The listing builds one solid part. Answer for the finished solid, in the listing's coordinates (mm). A direction names the side the tool comes from. Give positions to 0.01 mm unless a question says otherwise; leave off trailing zeros. Write each loop counter-clockwise with the first axis right and the second up, starting at its lowest first coordinate (ties: lowest second). Pieces come first, ordered by that corner, then holes. Notation, with made-up numbers: M 8.5,40 L 65.5,40 A19 ccw 65.5,66 Z; hole C 46,41.5 d7. An arc over 180 degrees is marked long. Return JSON: item names as keys, results as strings.
from build123d import *

# Parameters (mm, degrees)
FLANGE_PROFILE_R       = 12.5
FLANGE_PROFILE_R_2     = 12.920835642
FLANGE_PLATE_DEPTH     = 5
HUB_PROFILE_R          = 25
HUB_PROFILE_R_2        = 15
HUB_50_BORE_30_DEPTH   = 60
CROSS_SLOT_PROFILE_W   = 10
CROSS_SLOT_PROFILE_H   = 10.92
CROSS_SLOT_PROFILE_W_2 = 10.92
CROSS_SLOT_PROFILE_H_2 = 10
CROSS_SLOTS_4X10_DEPTH = 5


with BuildPart() as part:
    # Flange Profile → Flange Plate (new, symmetric)
    with BuildSketch(Plane(origin=(0, 0, 0), x_dir=(1, 0, 0), z_dir=(0, 1, 0))):
        with BuildLine():
            Line((-62.717391304, 19.30748114), (-9.130434783, 33.788091995))
            ThreePointArc((-9.130434783, 33.788091995), (0.242124563, 34.9991625), (9.597031237, 33.658535195))
            Line((9.597031237, 33.658535195), (57.5, 20))
            ThreePointArc((57.5, 20), (77.5, 0), (57.5, -20))
            Line((57.5, -20), (9.597031237, -33.658535195))
            ThreePointArc((9.597031237, -33.658535195), (0.242124563, -34.9991625), (-9.130434783, -33.788091995))
            Line((-9.130434783, -33.788091995), (-62.717391304, -19.30748114))
            ThreePointArc((-62.717391304, -19.30748114), (-77.5, 0), (-62.717391304, 19.30748114))
        make_face()
        with Locations(Location((-57.5, 0, 0), (0, 0, 270))):
            Circle(FLANGE_PROFILE_R, mode=Mode.SUBTRACT)
        with Locations(Location((57.5, 0, 0), (0, 0, 270))):
            Circle(FLANGE_PROFILE_R_2, mode=Mode.SUBTRACT)
    extrude(amount=FLANGE_PLATE_DEPTH, both=True)

    # Hub Profile → Hub Ø50 Bore Ø30 (add)
    with BuildSketch(Plane(origin=(0, 5, 0), x_dir=(1, 0, 0), z_dir=(0, 1, 0))):
        with Locations(Location((0, 0, 0), (0, 0, 270))):
            Circle(HUB_PROFILE_R)
        with Locations(Location((0, 0, 0), (0, 0, 270))):
            Circle(HUB_PROFILE_R_2, mode=Mode.SUBTRACT)
    extrude(amount=HUB_50_BORE_30_DEPTH)

    # Cross Slot Profile → Cross Slots 4x10 (cut)
    with BuildSketch(Plane(origin=(0, 65, 0), x_dir=(1, 0, 0), z_dir=(0, 1, 0))):
        with Locations((0, 19.602135624)):
            Rectangle(CROSS_SLOT_PROFILE_W, CROSS_SLOT_PROFILE_H)
        with Locations((19.602135624, 0)):
            Rectangle(CROSS_SLOT_PROFILE_W_2, CROSS_SLOT_PROFILE_H_2)
        with Locations((0, -19.602135624)):
            Rectangle(CROSS_SLOT_PROFILE_W, CROSS_SLOT_PROFILE_H)
        with Locations((-19.602135624, 0)):
            Rectangle(CROSS_SLOT_PROFILE_W_2, CROSS_SLOT_PROFILE_H_2)
    extrude(amount=-CROSS_SLOTS_4X10_DEPTH, mode=Mode.SUBTRACT)


solid = part.part
Item 1: A cutting plane is placed at C-C, the plane x = -57.5. Write down the section's boundary in (y, z).
Geometry results:
{"outline": "M -5,-20.72 L 5,-20.72 L 5,-12.5 L -5,-12.5 Z; M -5,12.5 L 5,12.5 L 5,20.72 L -5,20.72 Z"}
Item 2: Find the intervals of material crossed by line 1 (X direction, y = -3, z = 0); line 2 (X direction, y = 34, z = 0); line 3 (X direction, y = -1.5, z = 7.5), in increasing order.
Geometry results:
{"line 1": "x = -77.5 to -70, -45 to 44.58, 70.42 to 77.5", "line 2": "x = -25 to -15, 15 to 25", "line 3": "x = -76.04 to -67.5, -47.5 to 46.98, 68.02 to 76.04"}
Item 3: Given pin 1 Ø5.5 at (x, y) = (-20, 63) entering from +Z; pin 2 Ø4 at (y, z) = (63.5, 21) entering from -X; pin 3 Ø4 at (y, z) = (63, 19.5) entering from +X; pin 4 Ø3 at (x, z) = (-9.5, 10) entering from +Y, each flat-ended and moving along its own axis, determine where each tip first touches the part or whether it passes through.
Geometry results:
{"pin 1": "stops at z = 18.1", "pin 2": "stops at x = -16.25", "pin 3": "stops at x = 17.85", "pin 4": "stops at y = 65"}
Item 4: A cutting plane is placed at D-D, the plane y = 35. Write down the section's boundary in (x, z), plus the area to 3 significant figures.
Geometry results:
{"outline": "C 0,0 d50; hole C 0,0 d30", "area": "1,260 mm2"}
Item 5: Which of the six approach directions +Z, -Z, +X, -X, +Y, -Y give full straight-line access (tool end or side, diameter ignored) to faces 4 (the cylindrical face through (-13.31, 34.58, 6.92)), 5 (the cylindrical face through (-45.106, -0.07, -1.627)), 6 (the flat face through (0, 60, -20))?
Geometry results:
{"face 4": "+Y", "face 5": "+Y, -Y", "face 6": "+Z, -Z, +Y"}
Item 6: A cutting plane is placed at A-A, the plane y = 1.5. Write down the section's boundary in (x, z).
Geometry results:
{"outline": "M -62.72,-19.31 L -9.13,-33.79 A35 ccw 9.6,-33.66 L 57.5,-20 A20 ccw 57.5,20 L 9.6,33.66 A35 ccw -9.13,33.79 L -62.72,19.31 A20 ccw Z; hole C -57.5,0 d25; hole C 57.5,0 d25.84"}
Item 7: A cutting plane is placed at B-B, the plane z = 0. Write down the section's boundary in (x, y).
Geometry results:
{"outline": "M -77.5,-5 L -70,-5 L -70,5 L -77.5,5 Z; M -45,-5 L 44.58,-5 L 44.58,5 L 25,5 L 25,60 L 15,60 L 15,5 L -15,5 L -15,60 L -25,60 L -25,5 L -45,5 Z; M 70.42,-5 L 77.5,-5 L 77.5,5 L 70.42,5 Z"}
Item 8: Determine the mould class of faces 1 (the flat face through (-15, 65, -15)), 2 (the cylindrical face through (0, 0, 35)), 3 (the cylindrical face through (68.395, -0.07, 6.946)) for opening direction X: +X half, -X half, draft (parallel to the pull), parting line (faces both ways), or undercut.
Geometry results:
{"face 1": "draft", "face 2": "parting line", "face 3": "undercut"}
